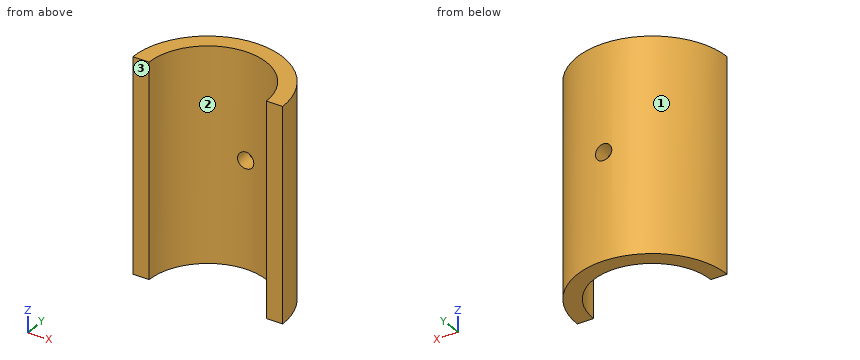
```python
from build123d import *

# Parameters (mm, degrees)
EXTRUDE_1_DEPTH    = 65
HOLE_WIZARD_M6_1_D = 5


with BuildPart() as part:
    # 草图1 → 凸台-拉伸1 (new body)
    with BuildSketch(Plane.XY):
        with BuildLine():
            Line((-23, 0), (-18, 0))
            ThreePointArc((-18, 0), (0, 18), (18, 0))
            Line((18, 0), (23, 0))
            ThreePointArc((23, 0), (0, 23), (-23, 0))
        make_face()
    extrude(amount=-EXTRUDE_1_DEPTH)

    # M6 螺纹孔1 (through all)
    with Locations(Plane(origin=(0, 23, -32.5), x_dir=(1, 0, 0), z_dir=(0, 1, 0))):
        with Locations((0, 0)):
            Hole(HOLE_WIZARD_M6_1_D / 2)


solid = part.part
```
The listing builds one solid part. Answer for the finished solid, in the listing's coordinates (mm). Face numbers are marked on the shaded views. Give positions to 0.01 mm unless a question says otherwise; leave off trailing zeros. Write each loop counter-clockwise with the first axis right and the second up, starting at its lowest first coordinate (ties: lowest second). Pieces come first, ordered by that corner, then holes. Notation, with made-up numbers: (46.25, 73.5) - (95.25, 73.5) arc R26 cw to (95.25, 97.5) - close; hole circle Ø9 at (76, 56). An arc over 180 degrees is marked (long way). Use one line per item in the form item = value. Start each with the question number.
1) Flat-ended cylindrical pins translate along their axes: pin 1 Ø1 at (x, y) = (11, 12) entering from -Z; pin 2 Ø4 at (x, z) = (7.5, -22) entering from -Y; pin 3 Ø1.5 at (y, z) = (12, -46) entering from +X; pin 4 Ø2 at (y, z) = (19.5, -42) entering from -X. Find the tip coordinate at first contact, or state that the pin passes through.
2) The mould has two halves that part along X. Classify the marked faces 1, 2 and 3: pulls with the +X half, pulls with the -X half, needs draft (parallel to the pull), parting line crosses it, or undercut.
3) Find section C-C on y = 19.75. Determine the outline of the cut face in (x, z), plus the area to 3 significant figures.
4) Find section B-B on z = -32.5. Determine the outline of the cut face in (x, y), plus the area to 3 significant figures.
5) Find section A-A on x = 0. Determine the outline of the cut face in (y, z).
6) Find section D-D on x = -11.5. Determine the outline of the cut face in (y, z), plus the area to 3 significant figures.
7) Consider line 1 along Z through (x, y) = (0, 21.6); line 2 along Y through (x, z) = (0, -22); line 3 along X through (y, z) = (8.25, -30). Determine where each line is inside the solid, lowest interval first. Write a range as from..to.
Geometry results:
q1.pin_1 = through
q1.pin_2 = 15.29
q1.pin_3 = 20.06
q1.pin_4 = -13.67
q2.face_1 = parting line crosses it
q2.face_2 = undercut
q2.face_3 = needs draft
q3.outline = (-11.79, -65) - (11.79, -65) - (11.79, 0) - (-11.79, 0) - close; hole circle Ø5 at (0, -32.5)
q3.area = 1,510 mm2
q4.outline = (-23, 0) - (-18, 0) arc R18 cw to (-2.5, 17.83) - (-2.5, 22.86) arc R23 ccw to start; (2.5, 17.83) arc R18 cw to (18, 0) - (23, 0) arc R23 ccw to (2.5, 22.86) - close
q4.area = 297 mm2
q5.outline = (18, -65) - (23, -65) - (23, -35) - (18, -35) - close; (18, -30) - (23, -30) - (23, 0) - (18, 0) - close
q6.outline = (13.85, -65) - (19.92, -65) - (19.92, 0) - (13.85, 0) - close
q6.area = 395 mm2
q7.line_1 = -65..-35, -30..0
q7.line_2 = 18..23
q7.line_3 = -21.47..-16, 16..21.47
